Geometry check sheet. Reference: the model listing, model coordinates, mm. A direction names the side the tool comes from. Give positions to 0.01 mm unless a question says otherwise; leave off trailing zeros. Loops run counter-clockwise (first coordinate to the right, second up) from the corner with the lowest first, then second, coordinate; pieces in that order, holes last. Notation, with made-up numbers: (16, 24.25) -> (75, 24.25) arc R24 ccw to (75, 46.25) -> close; hole circle Ø2 at (-13.75, 55). An arc over 180 degrees is marked (long way). One line per item, written item: value. Start each with the question number.
(1) Sectioned sample at C-C, the plane x = -133. Record the cut outline in (y, z).
(2) Sectioned sample at D-D, the plane x = 262. Record the cut outline in (y, z), then the cut area to 3 significant figures.
(3) Gauge pin test, flat ends, axial feed: pin 1 Ø6 at (x, y) = (-122.5, 40) entering from +Z; pin 2 Ø12 at (x, y) = (-319, 0.5) entering from +Z; pin 3 Ø12 at (x, z) = (-150, -38.5) entering from +Y. Record the tip position at first contact, or that the pin passes through.
(4) Scan lines: line 1 along X through (y, z) = (-1, 21.5); line 2 along X through (y, z) = (11, 32.5); line 3 along Y through (x, z) = (12, -2). Record each from-to range of solid material in increasing order. Write a range as from..to.
(5) Tool access check on faces 1 (the face through (-3.08, -32.26, -50.59)), 2 (the face through (-361.97, -13.38, 25.73)), 3 (the face through (360.53, -13.38, 25.73)). Record the directions out of +Z, -Z, +X, -X, +Y, -Y that give a thin tool (end or side, any length) a straight path to the whole face; none if there is none.
(6) Sectioned sample at A-A, the plane y = 0. Record the cut outline in (x, z), then the cut area to 3 significant figures.
from build123d import *

# Parameters (mm, degrees)
END_CHAMFER_7_5X45_SIZE = 7.5


with BuildPart() as part:
    # Shaft Profile Sketch → Stepped Shaft Body (revolve)
    with BuildSketch(Plane.XY, mode=Mode.PRIVATE) as stepped_shaft_body_sk:
        Polygon((220, 60), (-220, 60), (-220, 30), (-310, 30), (-310, 29), (-420, 29), (-420, 0), (420, 0), (420, 29), (310, 29), (310, 30), (220, 30), align=None)
    revolve(stepped_shaft_body_sk.sketch.rotate(Axis((-420, 0, 0), (1, 0, 0)), 180), axis=Axis((-420, 0, 0), (1, 0, 0)))

    # End Chamfer 7.5x45°
    end_chamfer_7_5x45_edges = [part.edges().sort_by_distance(p)[0] for p in [
        (-420, 29, 0),
        (420, 29, 0),
    ]]
    chamfer(end_chamfer_7_5x45_edges, length=END_CHAMFER_7_5X45_SIZE)


solid = part.part
Calculated:
1. outline: circle Ø120 at (0, 0)
2. outline: circle Ø60 at (0, 0)
2. area: 2,830 mm2
3. pin 1: stops at z = 47.23
3. pin 2: stops at z = 29
3. pin 3: stops at y = 50.44
4. line 1: x = -419.98..419.98
4. line 2: x = -220..220
4. line 3: y = -59.97..59.97
5. face 1: +X, -X
5. face 2: -X
5. face 3: +X
6. outline: (-420, -21.5) -> (-412.5, -29) -> (-310, -29) -> (-310, -30) -> (-220, -30) -> (-220, -60) -> (220, -60) -> (220, -30) -> (310, -30) -> (310, -29) -> (412.5, -29) -> (420, -21.5) -> (420, 21.5) -> (412.5, 29) -> (310, 29) -> (310, 30) -> (220, 30) -> (220, 60) -> (-220, 60) -> (-220, 30) -> (-310, 30) -> (-310, 29) -> (-412.5, 29) -> (-420, 21.5) -> close
6. area: 76,200 mm2
